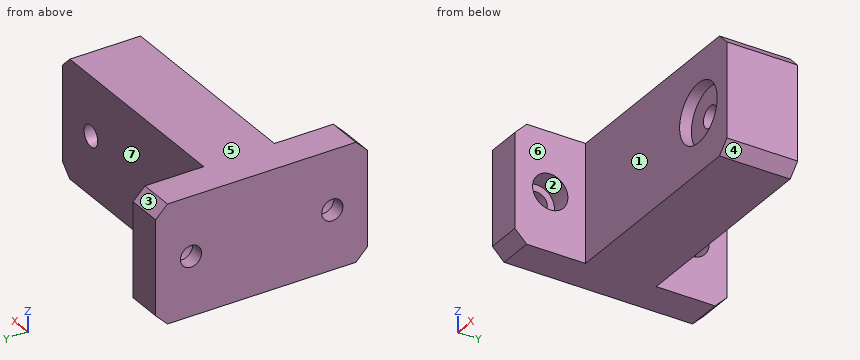
```python
from build123d import *

# Parameters (mm, degrees)
SKETCH_1_W                = 100
SKETCH_1_H                = 30
EXTRUDE_1_DEPTH           = 14
SKETCH_2_W                = 50
SKETCH_2_H                = 30
EXTRUDE_2_DEPTH           = 95
SKETCH_3_R                = 12.5
CUT_EXTRUDE_1_DEPTH       = 5
HOLE_WIZARD_9_0_9_1_D     = 9
HOLE_WIZARD_9_0_9_2_D     = 9
SKETCH_8_OUTSIDE_W        = 132.186
SKETCH_8_OUTSIDE_H        = 62.186
SKETCH_8_OUTSIDE_W_2      = 50
SKETCH_8_OUTSIDE_H_2      = 30
CUT_EXTRUDE_2_DEPTH       = 121.855285362
SKETCH_9_W                = 15
SKETCH_9_H                = 50
EXTRUDE_3_DEPTH           = 30
SKETCH_10_W               = 15
SKETCH_10_H               = 50
EXTRUDE_4_DEPTH           = 30
HOLE_WIZARD_1_D           = 9
HOLE_WIZARD_1_CBORE_D     = 15
HOLE_WIZARD_1_CBORE_DEPTH = 9
CHAMFER_1_SIZE            = 5


with BuildPart() as part:
    # 草图1 → 凸台-拉伸1 (new body)
    with BuildSketch(Plane(origin=(0, 0, 0), x_dir=(0, 0, -1), z_dir=(1, 0, 0))):
        Rectangle(SKETCH_1_W, SKETCH_1_H)
    extrude(amount=EXTRUDE_1_DEPTH)

    # 草图2 → 凸台-拉伸2 (add)
    with BuildSketch(Plane(origin=(14, 0, 0), x_dir=(0, 0, -1), z_dir=(1, 0, 0))):
        Rectangle(SKETCH_2_W, SKETCH_2_H)
    extrude(amount=EXTRUDE_2_DEPTH)

    # 草图3 → 切除-拉伸1 (cut)
    with BuildSketch(Plane.XZ.offset(15)):
        with Locations(Location((90, 0, 0), (0, 0, 270))):
            Circle(SKETCH_3_R)
    extrude(amount=-CUT_EXTRUDE_1_DEPTH, mode=Mode.SUBTRACT)

    # Ø9.0 (9) 直径孔1 (through all)
    with Locations(Plane(origin=(0, -15, 0), x_dir=(-1, 0, 0), z_dir=(0, -1, 0))):
        with Locations((-90, 0)):
            Hole(HOLE_WIZARD_9_0_9_1_D / 2)

    # Ø9.0 (9) 直径孔2 (through all)
    with Locations(Plane(origin=(14, 0, 0), x_dir=(0, 0, -1), z_dir=(1, 0, 0))):
        with Locations((-40, 0), (40, 0)):
            Hole(HOLE_WIZARD_9_0_9_2_D / 2)

    # 草图8 outside → 切除-拉伸2 (cut, through all)
    with BuildSketch(Plane(origin=(109, 0, 0), x_dir=(0, 0, -1), z_dir=(1, 0, 0))):
        Rectangle(SKETCH_8_OUTSIDE_W, SKETCH_8_OUTSIDE_H)
        Rectangle(SKETCH_8_OUTSIDE_W_2, SKETCH_8_OUTSIDE_H_2, mode=Mode.SUBTRACT)
    extrude(amount=-CUT_EXTRUDE_2_DEPTH, mode=Mode.SUBTRACT)

    # 草图9 → 凸台-拉伸3 (add)
    with BuildSketch(Plane.XZ.offset(15)):
        with Locations((7.5, 0)):
            Rectangle(SKETCH_9_W, SKETCH_9_H)
    extrude(amount=EXTRUDE_3_DEPTH)

    # 草图10 → 凸台-拉伸4 (add)
    with BuildSketch(Plane(origin=(0, 15, 0), x_dir=(1, 0, 0), z_dir=(0, 1, 0))):
        with Locations((7.5, 0)):
            Rectangle(SKETCH_10_W, SKETCH_10_H)
    extrude(amount=EXTRUDE_4_DEPTH)

    # 打孔尺寸(%根据)内六角圆柱头螺钉的类型1 (through all)
    with Locations(Plane(origin=(15, 0, 0), x_dir=(0, 0, -1), z_dir=(1, 0, 0))):
        with Locations((0, 30), (0, -30)):
            CounterBoreHole(HOLE_WIZARD_1_D / 2, HOLE_WIZARD_1_CBORE_D / 2, HOLE_WIZARD_1_CBORE_DEPTH)

    # 倒角1
    chamfer_1_edges = [part.edges().sort_by_distance(p)[0] for p in [
        (109, 0, -25),
        (109, 0, 25),
        (7.5, -45, -25),
        (7.5, -45, 25),
        (7.5, 45, 25),
        (7.5, 45, -25),
    ]]
    chamfer(chamfer_1_edges, length=CHAMFER_1_SIZE)


solid = part.part
```
Can you work these out from the model? Positions are in its coordinate system, mm. Face numbers are marked on the shaded views. A direction names the side the tool comes from. Coordinates: 2 decimals unless noted, no trailing zeros. Loops run counter-clockwise (first coordinate to the right, second up) from the corner with the lowest first, then second, coordinate; pieces in that order, holes last.
Item 1: Suppose I cut it at A-A (z = 0). State how many separate pieces and enclosed holes the cut face has, then the cut area to 3 significant figures.
Answers below:
separate pieces: 4
enclosed holes: 0
area: 3,440 mm2
Item 2: Please list where these lines run through material, in increasing order: L1, parallel to Y at x = 4, z = 0; L2, parallel to Y at x = 10.5, z = 0; L3, parallel to Z at x = 90, y = 1.75.
Answers below:
L1: y = -45 to -34.5, -25.5 to 25.5, 34.5 to 45
L2: y = -45 to -37.5, -22.5 to 22.5, 37.5 to 45
L3: z = -25 to -4.5, 4.5 to 25
Item 3: I'm going to push flat-ended pins straight in: pin 1 (15 mm diameter, centred on x = 55, z = -5.5, fed in from +Y); pin 2 (9 mm diameter, centred on y = 34.5, z = -5.5, fed in from +X); pin 3 (10.5 mm diameter, centred on y = -30, z = 0, fed in from +X). Where does each tip first touch, or does it pass through?
Answers below:
pin 1: stops at y = 15
pin 2: stops at x = 15
pin 3: stops at x = 6
Item 4: Which directions (+Z, -Z, +X, -X, +Y, -Y) give clear straight access to the entire face, cutting with the end or side of a thin tool? Please do the marked faces 5, 6 and 7.
Answers below:
face 5: +Z, +X, -X, +Y, -Y
face 6: +Z, -Z, +X, -Y
face 7: +Z, -Z, +X, +Y
Item 5: Suppose I cut it at D-D (y = -2). Please give me the cut outline in (x, z).
Answers below:
outline: (0, -25) - (104, -25) - (109, -20) - (109, 20) - (104, 25) - (0, 25) - close; hole circle Ø9 at (90, 0)
Item 6: Suppose I cut it at C-C (y = -30). Please give me the cut outline in (x, z).
Answers below:
outline: (0, -25) - (15, -25) - (15, -7.5) - (6, -7.5) - (6, -4.5) - (0, -4.5) - close; (0, 4.5) - (6, 4.5) - (6, 7.5) - (15, 7.5) - (15, 25) - (0, 25) - close
Item 7: Suppose I cut it at B-B (x = 90). Please give me the cut outline in (y, z), then the cut area to 3 significant figures.
Answers below:
outline: (-15, -25) - (15, -25) - (15, -4.5) - (-10, -4.5) - (-10, -12.5) - (-15, -12.5) - close; (-15, 12.5) - (-10, 12.5) - (-10, 4.5) - (15, 4.5) - (15, 25) - (-15, 25) - close
area: 1,150 mm2
Item 8: If we mould it in two halves opening along Z, with no side actions, what happens to the marked faces 1, 2, 3 and 4? For each: released by +Z, released by -Z, zero draft, split by the parting line, or undercut.
Answers below:
face 1: zero draft
face 2: undercut
face 3: released by +Z
face 4: released by -Z
